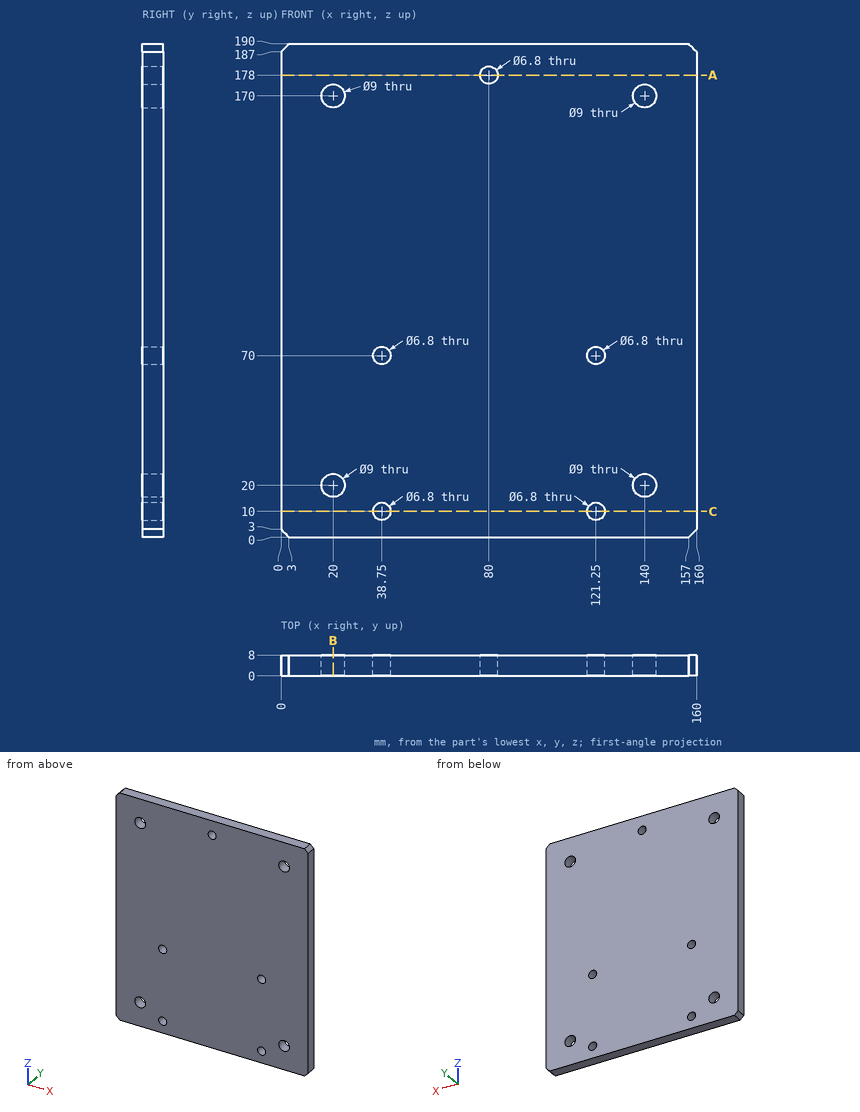
Can you work these out from the drawing? Everything is in mm from the part's minimum corner. Round coordinates to 2 decimals unless told otherwise and drop trailing zeros. Loops run counter-clockwise (first coordinate to the right, second up) from the corner with the lowest first, then second, coordinate; pieces in that order, holes last.
1. If I drill on line 1 along X through (y, z) = (5, 10); line 2 along Z through (x, y) = (140, 1.75); line 3 along X through (y, z) = (3, 170), over which ranges is the centre line in solid material (lowest first)?
Answer list:
line 1: x = 0 to 35.35, 42.15 to 117.85, 124.65 to 160
line 2: z = 0 to 15.5, 24.5 to 165.5, 174.5 to 190
line 3: x = 0 to 15.5, 24.5 to 135.5, 144.5 to 160
2. For P1, Ø5.5, axis at x = 121.25, z = 10, coming from the -Y side; P2, Ø11.5, axis at x = 20, z = 20, coming from the -Y side, each with a flat end and sliding along its axis, tell me the tip position at first contact or that it passes through.
Answer list:
P1: passes through
P2: stops at y = 0
3. If we section it at C-C on z = 10: Write out the boundary of the cut face in (x, y).
Answer list:
outline: (0, 0) - (35.35, 0) - (35.35, 8) - (0, 8) - close; (42.15, 0) - (117.85, 0) - (117.85, 8) - (42.15, 8) - close; (124.65, 0) - (160, 0) - (160, 8) - (124.65, 8) - close
4. If we section it at B-B on x = 20: Write out the boundary of the cut face in (y, z).
Answer list:
outline: (0, 0) - (8, 0) - (8, 15.5) - (0, 15.5) - close; (0, 24.5) - (8, 24.5) - (8, 165.5) - (0, 165.5) - close; (0, 174.5) - (8, 174.5) - (8, 190) - (0, 190) - close
5. If we section it at A-A on z = 178: Write out the boundary of the cut face in (x, y).
Answer list:
outline: (0, 0) - (76.6, 0) - (76.6, 8) - (0, 8) - close; (83.4, 0) - (160, 0) - (160, 8) - (83.4, 8) - close
